Could you check a few things on this model? Use its own coordinates, in mm. A direction names the side the tool comes from. Give positions to 0.01 mm unless a question says otherwise; leave off trailing zeros. Order: outer loops, then holes, each group sorted by start corner. A loop starts at its lowest first (then second) coordinate and runs counter-clockwise, first axis right, second up. Notation, with made-up numbers: (6.5, 27) - (29.5, 27) arc R6 ccw to (29.5, 34) - close; hole circle Ø9 at (-9, 13.25). An arc over 180 degrees is marked (long way). Put each result on its own line as item: value.
from build123d import *

# Parameters (mm, degrees)
SKETCH_1_R          = 4
EXTRUDE_1_DEPTH     = 6
SKETCH_2_R          = 1.4
CUT_EXTRUDE_1_DEPTH = 34.144531977
SKETCH_3_R          = 1
CUT_EXTRUDE_2_DEPTH = 5
SKETCH_4_W          = 4.960231778
SKETCH_4_H          = 1
EXTRUDE_2_DEPTH     = 6


with BuildPart() as part:
    # 草图1 → 凸台-拉伸1 (new body)
    with BuildSketch(Plane.XY):
        with BuildLine():
            Line((-23.6, 8), (23.6, 8))
            ThreePointArc((23.6, 8), (31.6, 0), (23.6, -8))
            Line((23.6, -8), (-23.6, -8))
            ThreePointArc((-23.6, -8), (-31.6, 0), (-23.6, 8))
        make_face()
        Circle(SKETCH_1_R, mode=Mode.SUBTRACT)
    extrude(amount=EXTRUDE_1_DEPTH)

    # 草图2 → 切除-拉伸1 (cut, through all)
    with BuildSketch(Plane.XY.offset(6)):
        with Locations((-23.6, 0)):
            Circle(SKETCH_2_R)
        with Locations((23.6, 0)):
            Circle(SKETCH_2_R)
    extrude(amount=-CUT_EXTRUDE_1_DEPTH, mode=Mode.SUBTRACT)

    # 草图3 → 切除-拉伸2 (cut)
    with BuildSketch(Plane(origin=(0, 8, 0), x_dir=(1, 0, 0), z_dir=(0, 1, 0))):
        with Locations(Location((0, -3, 0), (0, 0, 180))):
            Circle(SKETCH_3_R)
    extrude(amount=-CUT_EXTRUDE_2_DEPTH, mode=Mode.SUBTRACT)

    # 草图4 → 凸台-拉伸2 (add)
    with BuildSketch(Plane(origin=(0, 0, 0), x_dir=(-1, 0, 0), z_dir=(0, 0, -1))):
        with Locations((0, 4)):
            Rectangle(SKETCH_4_W, SKETCH_4_H)
    extrude(amount=-EXTRUDE_2_DEPTH)


solid = part.part
1) I'm going to push flat-ended pins straight in: pin 1 (5 mm diameter, centred on x = 0, y = 0, fed in from +Z); pin 2 (1.6 mm diameter, centred on x = 0, z = 3, fed in from +Y). Where does each tip first touch, or does it pass through?
Filled in:
pin 1: passes through
pin 2: stops at y = 4.5
2) We'd pull the mould along X, two halves only. Please class faces 4 (the flat face through (0, -8, 3)), 5 (the cylindrical face through (-31.598, -0.176, 2.958)), 6 (the flat face through (0, 4.5, 3)): pulls with the +X half, pulls with the -X half, needs draft (parallel to the pull), parting line crosses it, or undercut.
Filled in:
face 4: needs draft
face 5: pulls with the -X half
face 6: undercut
3) Which directions (+Z, -Z, +X, -X, +Y, -Y) give clear straight access to the entire face, cutting with the end or side of a thin tool? Please do faces 1 (the flat face through (0, 3.5, 3)), 2 (the cylindrical face through (0, 6, 4)), 3 (the flat face through (0, 4, 0)).
Filled in:
face 1: +Z, -Z
face 2: +Y
face 3: -Z, +X, -X, +Y, -Y
4) Suppose I cut it at A-A, the plane z = 4.7. List the corners of the cut face in (x, y) for me, and give its area (3 significant figures).
Filled in:
outline: (-23.6, -8) - (23.6, -8) arc R8 ccw to (23.6, 8) - (-23.6, 8) arc R8 ccw to start; hole circle Ø2.8 at (-23.6, 0); hole (-1.94, 3.5) arc R4 ccw (long way) to (1.94, 3.5) - close; hole circle Ø2.8 at (23.6, 0)
area: 895 mm^2
5) Suppose I cut it at B-B, the plane x = 0. List the corners of the cut face in (y, z) for me, and give its area (3 significant figures).
Filled in:
outline: (-8, 0) - (-4, 0) - (-4, 6) - (-8, 6) - close; (3.5, 0) - (8, 0) - (8, 2) - (4.5, 2) - (4.5, 4) - (8, 4) - (8, 6) - (3.5, 6) - close
area: 44.0 mm^2
6) If I drill on line 1 (X direction, y = -1.25, z = 0.8); line 2 (Y direction, x = -23.6, z = 2.35); line 3 (X direction, y = 3.25, z = 4.6), over which ranges is the centre line in solid material (lowest first)? Write a range as [from, to].
Filled in:
line 1: x = [-31.5, -24.23], [-22.97, -3.8], [3.8, 22.97], [24.23, 31.5]
line 2: y = [-8, -1.4], [1.4, 8]
line 3: x = [-30.91, -2.33], [2.33, 30.91]
